Verification items for the finished model (mm, model axes). Face numbers are marked on the shaded views. A direction names the side the tool comes from. Give positions to 0.01 mm unless a question says otherwise; leave off trailing zeros. Loops run counter-clockwise (first coordinate to the right, second up) from the corner with the lowest first, then second, coordinate; pieces in that order, holes last. Notation, with made-up numbers: (-37, -28) - (9, -28) arc R13 cw to (9, -24) - close; hole circle Ø5 at (0.25, 75). An arc over 180 degrees is marked (long way). Put each result on its own line as item: value. Start each with the question number.
```python
from build123d import *

# Parameters (mm, degrees)
FILLET_1_R          = 0.5
CHAMFER_1_SIZE      = 0.866025404
CHAMFER_1_SIZE2     = 0.5
SKETCH_2_R          = 0.87
CUT_EXTRUDE_1_DEPTH = 500


with BuildPart() as part:
    # 草图1 → Revolve 700 (revolve)
    with BuildSketch(Plane.XY, mode=Mode.PRIVATE) as revolve_700_sk:
        with BuildLine():
            Line((0, 0), (31.5, 0))
            Line((31.5, 0), (31.5, 2))
            Line((31.5, 2), (1.5, 2))
            Line((1.5, 2), (1.5, 2.25))
            ThreePointArc((1.5, 2.25), (0.75, 3), (0, 2.25))
            Line((0, 2.25), (0, 0))
        make_face()
    revolve(revolve_700_sk.sketch.rotate(Axis((0, 0, 0), (1, 0, 0)), 90), axis=Axis((0, 0, 0), (1, 0, 0)))

    # 圆角1
    fillet_1_edges = [part.edges().sort_by_distance(p)[0] for p in [
        (1.5, 0, -2),
    ]]
    fillet(fillet_1_edges, radius=FILLET_1_R)

    # 倒角1
    chamfer_1_edges = [part.edges().sort_by_distance(p)[0] for p in [
        (31.5, 0, -2),
    ]]
    chamfer_1_side = [part.faces().sort_by_distance(p)[0] for p in [
        (16.737372436, 0, -2),
    ]]
    chamfer(chamfer_1_edges, length=CHAMFER_1_SIZE, length2=CHAMFER_1_SIZE2, reference=chamfer_1_side[0])

    # 草图2 → 切除-拉伸1 (cut, symmetric)
    with BuildSketch(Plane(origin=(0, 0, 0), x_dir=(1, 0, 0), z_dir=(0, 1, 0))):
        with Locations(Location((28.5, 0, 0), (0, 0, 270))):
            Circle(SKETCH_2_R)
    extrude(amount=CUT_EXTRUDE_1_DEPTH, both=True, mode=Mode.SUBTRACT)


solid = part.part
```
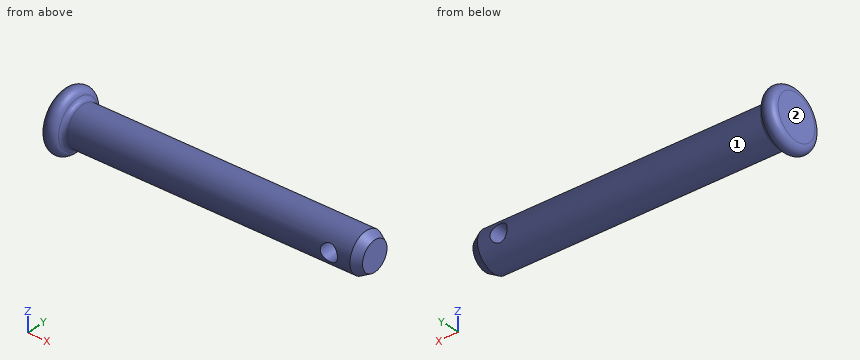
1) Depth check by flat-ended pin: P1, Ø1.5, axis at x = 19, z = 0.5, coming from the -Y side; P2, Ø1, axis at x = 17.5, y = -1, coming from the +Z side; P3, Ø2, axis at y = 2, z = 1.5, coming from the -X side. Enter the tip coordinate at first touch or a pass-through.
2) Scan lines: line 1 along X through (y, z) = (-0.85, 0); line 2 along Y through (x, z) = (18.5, 0); line 3 along Z through (x, y) = (28, -0.25). Record each from-to range of solid material in increasing order. Write a range as from..to.
3) Section check B-B, the plane x = 28.5. Enter the section's corners in (y, z), plus the area to 3 significant figures.
4) Section check A-A, the plane x = 12. Enter the section's corners in (y, z).
5) Set-up check for the marked faces 1 and 2: record each of +Z, -Z, +X, -X, +Y, -Y from which the full face is reachable in a straight line by a thin tool's end or side.
Results are:
1. P1: stops at y = -2
1. P2: stops at z = 1.94
1. P3: stops at x = 0
2. line 1: x = 0..27.63, 29.37..31.5
2. line 2: y = -2..2
2. line 3: z = -1.98..-0.71, 0.71..1.98
3. outline: (-1.8, -0.87) arc R2 ccw to (1.8, -0.87) - close; (-1.8, 0.87) - (1.8, 0.87) arc R2 ccw to start
3. area: 5.83 mm2
4. outline: circle Ø4 at (0, 0)
5. face 1: +X
5. face 2: +Z, -Z, -X, +Y, -Y
